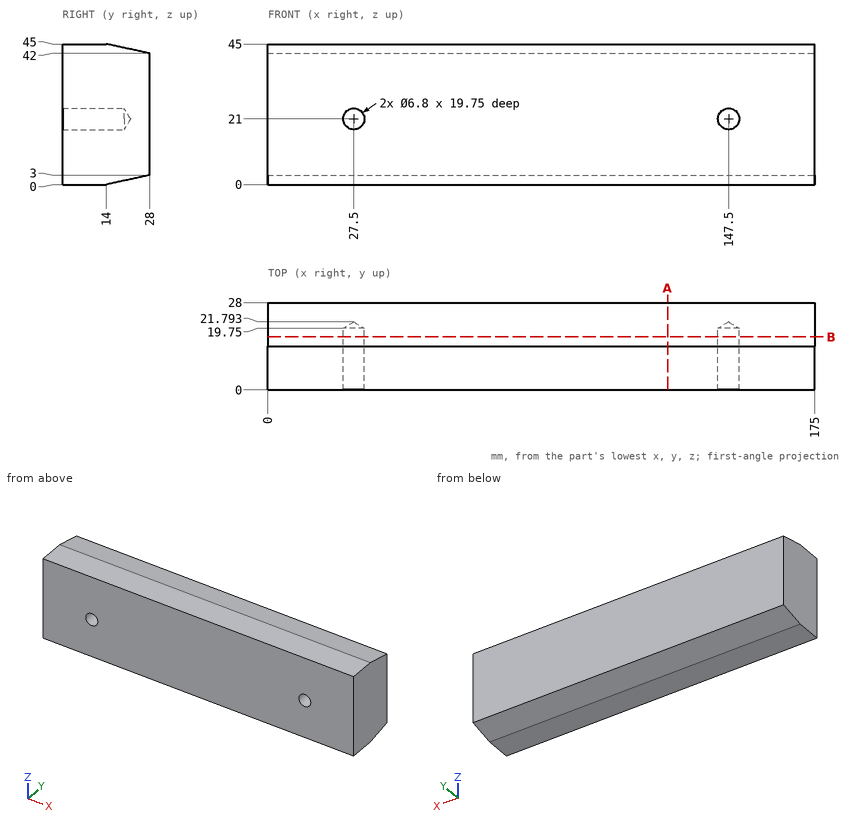
Geometry check sheet. Reference: drawing and pictorial views, mm from the part's lowest x, y, z. Round coordinates to 2 decimals unless told otherwise and drop trailing zeros. Write each loop counter-clockwise with the first axis right and the second up, starting at its lowest first coordinate (ties: lowest second). Pieces come first, ordered by that corner, then holes.
(1) Section check A-A (x = 128). Enter the section's corners in (y, z), plus the area to 3 significant figures.
Returned:
outline: (0, 0) - (14, 0) - (28, 3) - (28, 42) - (14, 45) - (0, 45) - close
area: 1,220 mm2
(2) Material ranges on line 1 (X direction, y = 9.75, z = 21); line 2 (Z direction, x = 27.5, y = 12.75); line 3 (Z direction, x = 89, y = 20), recorded low to high.
Returned:
line 1: x = 0 to 24.1, 30.9 to 144.1, 150.9 to 175
line 2: z = 0 to 17.6, 24.4 to 45
line 3: z = 1.29 to 43.71
(3) Depth check by flat-ended pin: pin 1 Ø2 at (y, z) = (23, 22.5) entering from -X. Enter the tip coordinate at first touch or a pass-through.
Returned:
pin 1: stops at x = 0
(4) Section check B-B (y = 17). Enter the section's corners in (x, z).
Returned:
outline: (0, 0.64) - (175, 0.64) - (175, 44.36) - (0, 44.36) - close; hole circle Ø6.8 at (27.5, 21); hole circle Ø6.8 at (147.5, 21)
